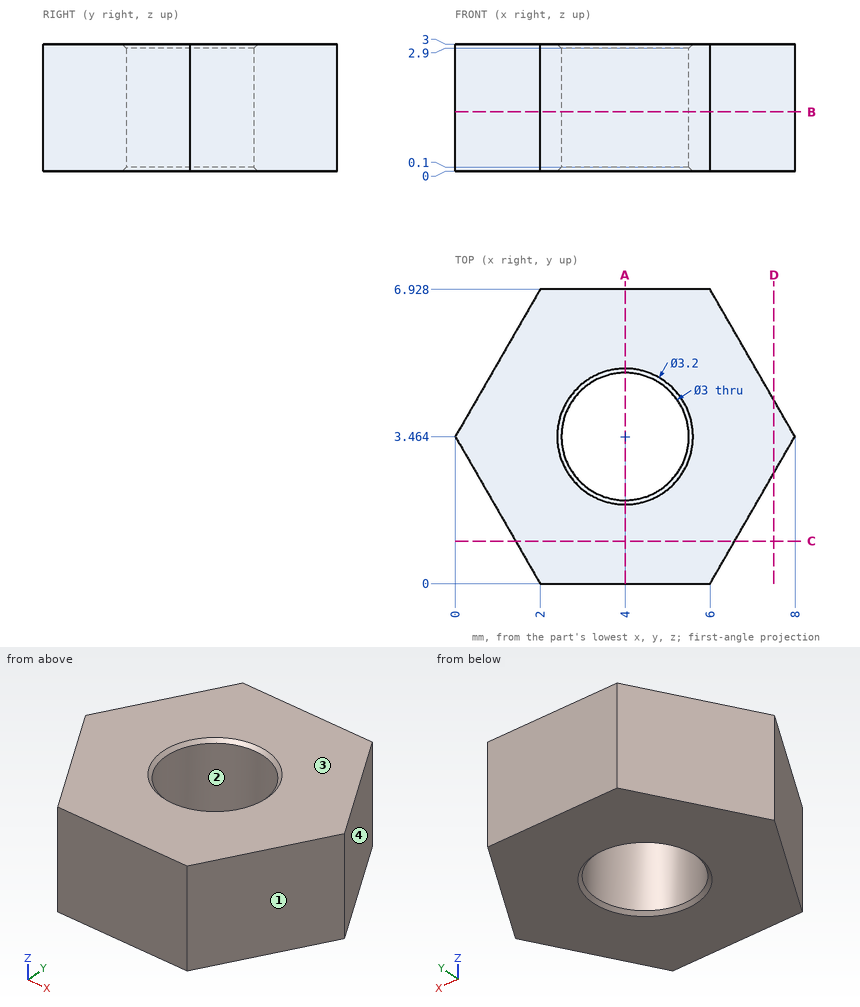
Can you work these out from the drawing? Everything is in mm from the part's minimum corner. Give positions to 0.01 mm unless a question says otherwise; leave off trailing zeros. Loops run counter-clockwise (first coordinate to the right, second up) from the corner with the lowest first, then second, coordinate; pieces in that order, holes last. Notation, with made-up numbers: (12, 74.25) -> (48, 74.25) arc R13 ccw to (48, 80.25) -> close; hole circle Ø4 at (-7.75, -7). An arc over 180 degrees is marked (long way). Put each result on its own line as item: value.
(1) Imagine slicing it at A-A on x = 4. Write out the boundary of the cut face in (y, z), plus the area to 3 significant figures.
Computed:
outline: (0, 0) -> (1.86, 0) -> (1.96, 0.1) -> (1.96, 2.9) -> (1.86, 3) -> (0, 3) -> close; (4.96, 0.1) -> (5.06, 0) -> (6.93, 0) -> (6.93, 3) -> (5.06, 3) -> (4.96, 2.9) -> close
area: 11.8 mm^2
(2) Thinking about a two-plate mould opening in Y: for the marked faces 1, 2, 3 and 4, which applies, pulls with the +Y half, pulls with the -Y half, needs draft (parallel to the pull), parting line crosses it, or undercut?
Computed:
face 1: pulls with the -Y half
face 2: undercut
face 3: needs draft
face 4: pulls with the +Y half
(3) Imagine slicing it at C-C on y = 1. Write out the boundary of the cut face in (x, z).
Computed:
outline: (1.42, 0) -> (6.58, 0) -> (6.58, 3) -> (1.42, 3) -> close
(4) I'm going to push flat-ended pins straight in: pin 1 Ø1 at (x, y) = (1.5, 3.5) entering from -Z; pin 2 Ø2.5 at (x, y) = (4, 3.46) entering from -Z. Where does each tip first touch, or does it pass through?
Computed:
pin 1: z = 0
pin 2: through
(5) Imagine slicing it at B-B on z = 1.4. Write out the boundary of the cut face in (x, y), plus the area to 3 significant figures.
Computed:
outline: (0, 3.46) -> (2, 0) -> (6, 0) -> (8, 3.46) -> (6, 6.93) -> (2, 6.93) -> close; hole circle Ø3 at (4, 3.46)
area: 34.5 mm^2
(6) Please list where these lines run through material, in increasing order: probe 1 along Y at (x, z) = (4, 0.8); probe 2 along X at (y, z) = (3.75, 2.85) (1 decimal); probe 3 along X at (y, z) = (3, 1.7). Write a range as [from, to].
Computed:
probe 1: [0, 1.96], [4.96, 6.93]
probe 2: [0.2, 2.5], [5.5, 7.8]
probe 3: [0.27, 2.57], [5.43, 7.73]
(7) Imagine slicing it at D-D on x = 7.5. Write out the boundary of the cut face in (y, z).
Computed:
outline: (2.6, 0) -> (4.33, 0) -> (4.33, 3) -> (2.6, 3) -> close
